Geometry: see drawing. Coordinates: mm, zero at the bounding-box minimum. A direction names the side the tool comes from. Coordinates: 2 decimals unless noted, no trailing zeros. Loops run counter-clockwise (first coordinate to the right, second up) from the corner with the lowest first, then second, coordinate; pieces in that order, holes last. Notation, with made-up numbers: (22.5, 39) - (47.5, 39) arc R18 ccw to (47.5, 69) - close; hole circle Ø1 at (5, 64). An arc over 180 degrees is marked (long way). Answer in a Markdown table with one row per item.
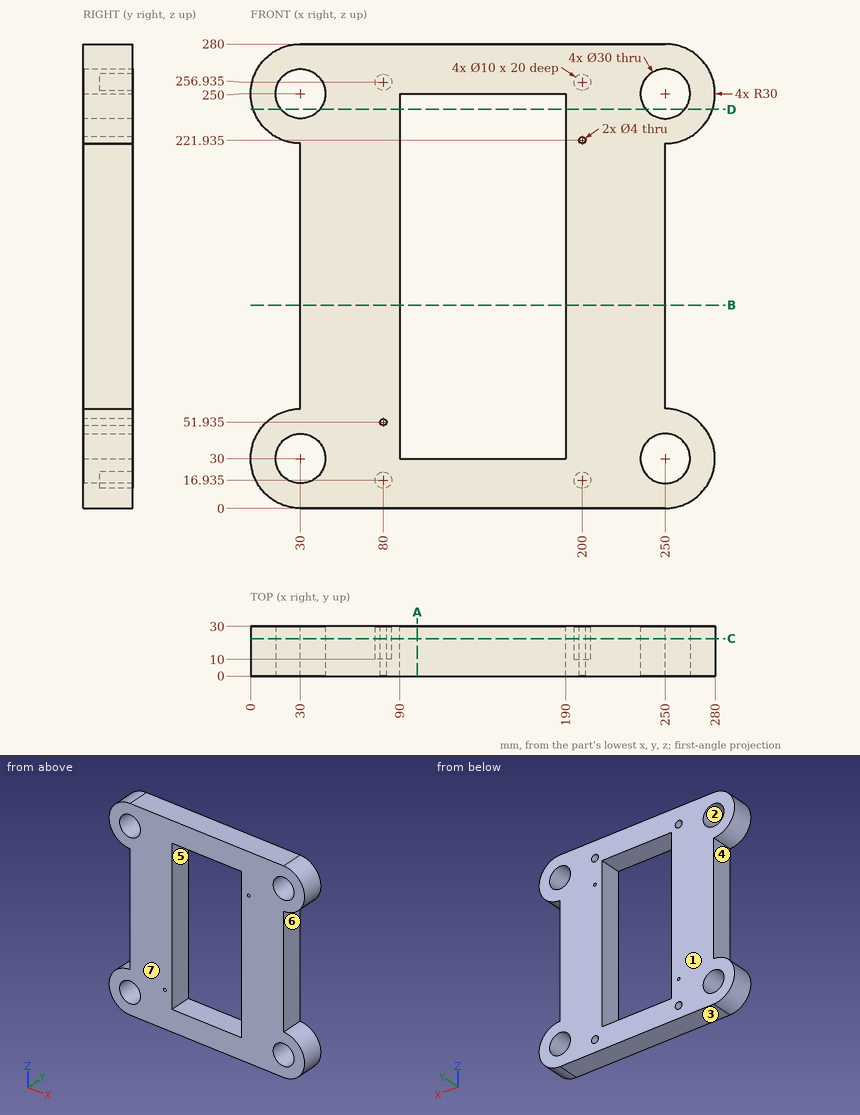
(1) First-contact query: pin 1 Ø6 at (y, z) = (6.5, 114) entering from -X; pin 2 Ø3 at (y, z) = (11, 40) entering from +X; pin 3 Ø5 at (x, z) = (78, 256) entering from +Y. Flat tips, straight axial feed; report the tip coordinate or a pass-through.
Verdict:
| item | result |
|---|---|
| pin 1 | stops at x = 30 |
| pin 2 | stops at x = 278.77 |
| pin 3 | stops at y = 10 |
(2) Cut plane C-C on y = 22.5. State how many separate pieces and enclosed holes the cut face has, then the cut area to 3 significant figures.
Verdict:
| item | result |
|---|---|
| separate pieces | 1 |
| enclosed holes | 11 |
| area | 42,100 mm² |
(3) Ray query, probe 1 along Z at (x, y) = (200.5, 26.5); probe 2 along Z at (x, y) = (129, 24.25); probe 3 along X at (y, z) = (21.5, 258.5). Return the intervals inside material, ascending.
Verdict:
| item | result |
|---|---|
| probe 1 | z = 0 to 11.96, 21.91 to 220, 223.87 to 251.96, 261.91 to 280 |
| probe 2 | z = 0 to 30, 250 to 280 |
| probe 3 | x = 1.23 to 17.64, 42.36 to 75.25, 84.75 to 195.25, 204.75 to 237.64, 262.36 to 278.77 |
(4) Cut plane A-A on x = 100.5. Output: boundary loops of the cut face in (y, z).
Verdict:
| item | result |
|---|---|
| outline | (0, 0) - (30, 0) - (30, 30) - (0, 30) - close; (0, 250) - (30, 250) - (30, 280) - (0, 280) - close |
(5) Cut plane B-B on z = 122.5. Output: boundary loops of the cut face in (x, y), then the cut area to 3 significant figures.
Verdict:
| item | result |
|---|---|
| outline | (30, 0) - (90, 0) - (90, 30) - (30, 30) - close; (190, 0) - (250, 0) - (250, 30) - (190, 30) - close |
| area | 3,600 mm² |
(6) Cut plane D-D on z = 240.5. Output: boundary loops of the cut face in (x, y), then the cut area to 3 significant figures.
Verdict:
| item | result |
|---|---|
| outline | (1.54, 0) - (18.39, 0) - (18.39, 30) - (1.54, 30) - close; (41.61, 0) - (90, 0) - (90, 30) - (41.61, 30) - close; (190, 0) - (238.39, 0) - (238.39, 30) - (190, 30) - close; (261.61, 0) - (278.46, 0) - (278.46, 30) - (261.61, 30) - close |
| area | 3,910 mm² |
(7) Access query for the marked faces 4, 5, 6 and 7. Directions: +Z, -Z, +X, -X, +Y, -Y. A direction counts if a zero-diameter tool reaches every point of the face in a straight line with its end or side. Return the directions, or none.
Verdict:
| item | result |
|---|---|
| face 4 | -X, +Y, -Y |
| face 5 | +Y, -Y |
| face 6 | +X, +Y, -Y |
| face 7 | +Z, -Z, +X, -X, -Y |
(8) Pull-direction query (Z, two-part tool) for the marked faces 1, 2 and 3; classes: pulls with the +Z half, pulls with the -Z half, needs draft (parallel to the pull), parting line crosses it, or undercut.
Verdict:
| item | result |
|---|---|
| face 1 | needs draft |
| face 2 | undercut |
| face 3 | pulls with the -Z half |
